```python
from build123d import *

# Parameters (mm, degrees)
SKETCH1_R           = 2
BOSS_EXTRUDE1_DEPTH = 10


with BuildPart() as part:
    # Sketch1 → Boss-Extrude1 (new body)
    with BuildSketch(Plane(origin=(0, 0, 0), x_dir=(1, 0, 0), z_dir=(0, 1, 0))):
        with BuildLine():
            Line((-125, 4), (125, 4))
            ThreePointArc((125, 4), (129, 0), (125, -4))
            Line((125, -4), (-125, -4))
            ThreePointArc((-125, -4), (-129, 0), (-125, 4))
        make_face()
        with Locations(Location((-125, 0, 0), (0, 0, 270))):
            Circle(SKETCH1_R, mode=Mode.SUBTRACT)
        with Locations(Location((125, 0, 0), (0, 0, 270))):
            Circle(SKETCH1_R, mode=Mode.SUBTRACT)
    extrude(amount=BOSS_EXTRUDE1_DEPTH)


solid = part.part
```
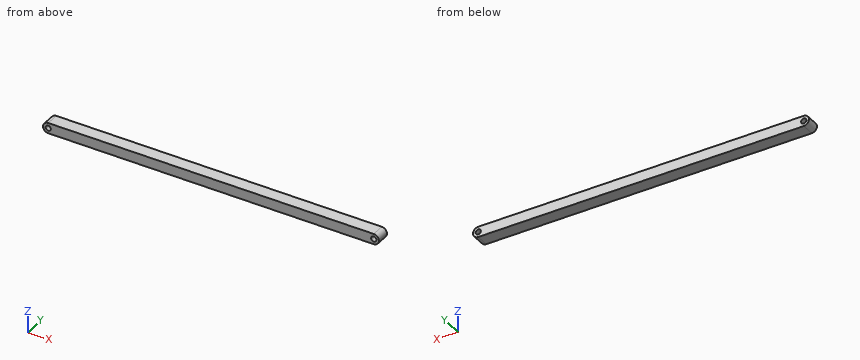
Source: CAD feature listing. Evaluate the final solid. Frame: model axes, mm. Round coordinates to 2 decimals unless told otherwise and drop trailing zeros. Loops run counter-clockwise (first coordinate to the right, second up) from the corner with the lowest first, then second, coordinate; pieces in that order, holes last.
1. Section query B-B on y = 6.75. Output: boundary loops of the cut face in (x, z).
2. Ray query, L1, parallel to X at y = 4, z = 0; L2, parallel to X at y = 9, z = 1.5; L3, parallel to X at y = 3.5, z = -2.75. Return the intervals inside material, ascending.
3. Section query A-A on z = 0. Output: boundary loops of the cut face in (x, y).
Answers below:
1. outline: (-125, -4) - (125, -4) arc R4 ccw to (125, 4) - (-125, 4) arc R4 ccw to start; hole circle Ø4 at (-125, 0); hole circle Ø4 at (125, 0)
2. L1: x = -129 to -127, -123 to 123, 127 to 129
2. L2: x = -128.71 to -126.32, -123.68 to 123.68, 126.32 to 128.71
2. L3: x = -127.9 to 127.9
3. outline: (-129, 0) - (-127, 0) - (-127, 10) - (-129, 10) - close; (-123, 0) - (123, 0) - (123, 10) - (-123, 10) - close; (127, 0) - (129, 0) - (129, 10) - (127, 10) - close
